```python
from build123d import *

# Parameters (mm, degrees)
SKETCH1_W           = 100
SKETCH1_H           = 70
BOSS_EXTRUDE1_DEPTH = 8
FILLET1_R           = 10
SKETCH2_R           = 7
CUT_EXTRUDE1_DEPTH  = 8


with BuildPart() as part:
    # Sketch1 → Boss-Extrude1 (new body)
    with BuildSketch(Plane(origin=(0, 0, 0), x_dir=(1, 0, 0), z_dir=(0, 1, 0))):
        Rectangle(SKETCH1_W, SKETCH1_H)
    extrude(amount=BOSS_EXTRUDE1_DEPTH)

    # Fillet1
    fillet1_edges = [part.edges().sort_by_distance(p)[0] for p in [
        (-50, 4, -35),
        (50, 4, -35),
        (50, 4, 35),
        (-50, 4, 35),
    ]]
    fillet(fillet1_edges, radius=FILLET1_R)

    # Sketch2 → Cut-Extrude1 (cut)
    with BuildSketch(Plane(origin=(0, 8, 0), x_dir=(1, 0, 0), z_dir=(0, 1, 0))):
        with Locations(Location((-30, 0, 0), (0, 0, 270))):
            Circle(SKETCH2_R)
    extrude(amount=-CUT_EXTRUDE1_DEPTH, mode=Mode.SUBTRACT)


solid = part.part
```
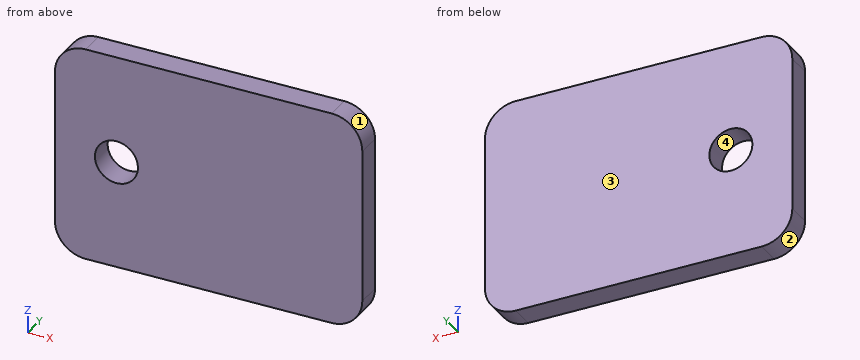
Read the model definition and answer for the solid it produces. Units are mm, in the model's axes. Face numbers are marked on the shaded views. Give positions to 0.01 mm unless a question says otherwise; leave off trailing zeros. Order: outer loops, then holes, each group sorted by start corner. A loop starts at its lowest first (then second) coordinate and runs counter-clockwise, first axis right, second up. Notation, with made-up numbers: (-36, 63.5) -> (19, 63.5) arc R20 ccw to (19, 91.5) -> close; hole circle Ø10 at (10.25, 26.5). An arc over 180 degrees is marked (long way). One line per item, written item: value. Start each with the question number.
(1) Straight lines are drawn through the part: L1, parallel to X at y = 5.75, z = 0; L2, parallel to Z at x = -29.5, y = 6; L3, parallel to Z at x = 40.5, y = 7.75. For each, find the intervals that lie inside material, in ascending order.
(2) The part is cut by section C-C (y = 5.25). Determine the outline of the cut face in (x, z), and give its area (3 significant figures).
(3) The part is cut by section A-A (z = 0). Determine the outline of the cut face in (x, y), and give its area (3 significant figures).
(4) For a pull along X with two mould halves and no side action, classify the marked faces 1, 2, 3 and 4 as released by +X, released by -X, zero draft, split by the parting line, or undercut.
(5) The part is cut by section B-B (x = -30). Determine the outline of the cut face in (y, z).
Taken from the geometry:
1. L1: -50 to -37, -23 to 50
1. L2: -35 to -6.98, 6.98 to 35
1. L3: -34.99 to 34.99
2. outline: (-50, -25) arc R10 ccw to (-40, -35) -> (40, -35) arc R10 ccw to (50, -25) -> (50, 25) arc R10 ccw to (40, 35) -> (-40, 35) arc R10 ccw to (-50, 25) -> close; hole circle Ø14 at (-30, 0)
2. area: 6,760 mm^2
3. outline: (-50, 0) -> (-37, 0) -> (-37, 8) -> (-50, 8) -> close; (-23, 0) -> (50, 0) -> (50, 8) -> (-23, 8) -> close
3. area: 688 mm^2
4. face 1: released by +X
4. face 2: released by -X
4. face 3: zero draft
4. face 4: undercut
5. outline: (0, -35) -> (8, -35) -> (8, -7) -> (0, -7) -> close; (0, 7) -> (8, 7) -> (8, 35) -> (0, 35) -> close
